from build123d import *

# Parameters (mm, degrees)
BOSS_EXTRUDE_1_DEPTH = 20
BOSS_EXTRUDE_2_DEPTH = 20
BOSS_EXTRUDE_START   = 58
SKETCH_3_R           = 25
BOSS_EXTRUDE_3_DEPTH = 40


with BuildPart() as part:
    # Sketch 1 → Boss-Extrude 1 (new body)
    with BuildSketch(Plane(origin=(0, 0, 0), x_dir=(1, 0, 0), z_dir=(0, 1, 0))):
        with BuildLine():
            Line((113, 90), (-113, 90))
            ThreePointArc((-113, 90), (-121.485281374, 86.485281374), (-125, 78))
            Line((-125, 78), (-125, -78))
            ThreePointArc((-125, -78), (-121.485281374, -86.485281374), (-113, -90))
            Line((-113, -90), (113, -90))
            ThreePointArc((113, -90), (121.485281374, -86.485281374), (125, -78))
            Line((125, -78), (125, 78))
            ThreePointArc((125, 78), (121.485281374, 86.485281374), (113, 90))
        make_face()
    extrude(amount=BOSS_EXTRUDE_1_DEPTH)

    # Sketch 2 → Boss-Extrude 2 (add)
    with BuildSketch(Plane.XZ):
        with BuildLine():
            Line((48, 80), (-48, 80))
            ThreePointArc((-48, 80), (-49.414213562, 79.414213562), (-50, 78))
            Line((-50, 78), (-50, -78))
            ThreePointArc((-50, -78), (-49.414213562, -79.414213562), (-48, -80))
            Line((-48, -80), (48, -80))
            ThreePointArc((48, -80), (49.414213562, -79.414213562), (50, -78))
            Line((50, -78), (50, 78))
            ThreePointArc((50, 78), (49.414213562, 79.414213562), (48, 80))
        make_face()
    extrude(amount=BOSS_EXTRUDE_2_DEPTH)

    # Sketch 3 → Boss-Extrude 3 (add)
    with BuildSketch(Plane(origin=(0, 0, 0), x_dir=(0, 0, -1), z_dir=(1, 0, 0)).offset(BOSS_EXTRUDE_START)):
        with BuildLine():
            Line((-59.224993899, 209.61249695), (-90, 20))
            Line((-90, 20), (90, 20))
            Line((90, 20), (59.224993899, 209.61249695))
            ThreePointArc((59.224993899, 209.61249695), (0, 260), (-59.224993899, 209.61249695))
        make_face()
        with Locations((0, 200)):
            Circle(SKETCH_3_R, mode=Mode.SUBTRACT)
    boss_extrude_3 = extrude(amount=BOSS_EXTRUDE_3_DEPTH)

    # Mirror 1: Boss-Extrude 3 across plane
    add(boss_extrude_3.mirror(Plane(origin=(0, 0, 0), x_dir=(0, 0, 1), z_dir=(1, 0, 0))))


solid = part.part
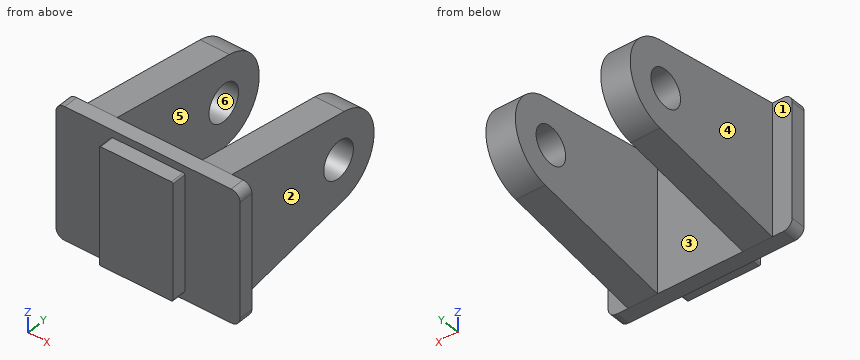
The listing builds one solid part. Answer for the finished solid, in the listing's coordinates (mm). Face numbers are marked on the shaded views. A direction names the side the tool comes from. Coordinates: 2 decimals unless noted, no trailing zeros. Write each loop counter-clockwise with the first axis right and the second up, starting at its lowest first coordinate (ties: lowest second). Pieces come first, ordered by that corner, then holes. Notation, with made-up numbers: M -20,43 L -9,43 A15 ccw -9,52 Z; hole C 49,20 d10. An arc over 180 degrees is marked long. Put each result on its own line as item: value. Start each with the question number.
1. Which of the six approach directions +Z, -Z, +X, -X, +Y, -Y give full straight-line access (tool end or side, diameter ignored) to the marked faces 4, 5 and 6?
2. A cutting plane is placed at A-A on x = 75. Write down the section's boundary in (y, z) (1 decimal).
3. Consider line 1 (X direction, y = 158.5, z = 15); line 2 (Y direction, x = -83, z = 0); line 3 (Y direction, x = 112, z = 13). Determine where each line is inside the solid, lowest interval first. Write a range as from..to.
4. A cutting plane is placed at D-D on y = 29. Write down the section's boundary in (x, z), then the cut area to 3 significant figures.
5. A cutting plane is placed at C-C on y = 200. Write down the section's boundary in (x, z), then the cut area to 3 significant figures.
6. Flat-ended cylindrical pins translate along their axes: P1, Ø8, axis at y = 132, z = -47, coming from the -X side; P2, Ø1, axis at x = -73, z = 3.5, coming from the -Y side; P3, Ø22, axis at y = -14.5, z = -5.5, coming from the +X side; P4, Ø10, axis at x = -10, y = 27.5, coming from the +Z side. Find the tip coordinate at first contact, or state that the pin passes through.
7. A cutting plane is placed at B-B on z = 0. Write down the section's boundary in (x, y).
8. For a pull along X with two mould halves and no side action, classify the marked faces 1, 2 and 3 as pulls with the +X half, pulls with the -X half, needs draft (parallel to the pull), parting line crosses it, or undercut.
Resolved:
1. face 4: +Z, -Z, -X, +Y
1. face 5: +Z, -Z, +Y
1. face 6: +X, -X
2. outline: M 0,-90 L 20,-90 L 209.6,-59.2 A60 ccw 209.6,59.2 L 20,90 L 0,90 Z; hole C 200,0 d50
3. line 1: x = -98..-58, 58..98
3. line 2: y = 0..175, 225..260
3. line 3: y = 0..20
4. outline: M -98,-88.54 L -58,-88.54 L -58,88.54 L -98,88.54 Z; M 58,-88.54 L 98,-88.54 L 98,88.54 L 58,88.54 Z
4. area: 14,200 mm2
5. outline: M -98,-60.79 L -58,-60.79 L -58,-25 L -98,-25 Z; M -98,25 L -58,25 L -58,60.79 L -98,60.79 Z; M 58,-60.79 L 98,-60.79 L 98,-25 L 58,-25 Z; M 58,25 L 98,25 L 98,60.79 L 58,60.79 Z
5. area: 5,730 mm2
6. P1: stops at x = -98
6. P2: stops at y = 0
6. P3: stops at x = 50
6. P4: passes through
7. outline: M -125,0 L -50,0 L -50,-20 L 50,-20 L 50,0 L 125,0 L 125,20 L 98,20 L 98,175 L 58,175 L 58,20 L -58,20 L -58,175 L -98,175 L -98,20 L -125,20 Z; M -98,225 L -58,225 L -58,260 L -98,260 Z; M 58,225 L 98,225 L 98,260 L 58,260 Z
8. face 1: needs draft
8. face 2: pulls with the +X half
8. face 3: undercut
